```python
from build123d import *

# Parameters (mm, degrees)
SKETCH_1_R          = 10
EXTRUDE_1_DEPTH     = 377.5
SKETCH_2_W          = 20.903935991
SKETCH_2_H          = 21
CUT_EXTRUDE_1_DEPTH = 25
CUT_EXTRUDE_START   = -30
SKETCH_5_R          = 10
SKETCH_5_R_2        = 9.5
CUT_EXTRUDE_2_DEPTH = 1.1


with BuildPart() as part:
    # 草图1 → 凸台-拉伸1 (new, symmetric)
    with BuildSketch(Plane.XY):
        Circle(SKETCH_1_R)
    extrude(amount=EXTRUDE_1_DEPTH, both=True)

    # 草图2 → 切除-拉伸1 (cut, symmetric)
    with BuildSketch(Plane(origin=(0, 0, 0), x_dir=(1, 0, 0), z_dir=(0, 1, 0))):
        with Locations((-17.951967996, 367)):
            Rectangle(SKETCH_2_W, SKETCH_2_H)
        with Locations((17.951967996, 367)):
            Rectangle(SKETCH_2_W, SKETCH_2_H)
        with Locations((17.951967996, -367)):
            Rectangle(SKETCH_2_W, SKETCH_2_H)
        with Locations((-17.951967996, -367)):
            Rectangle(SKETCH_2_W, SKETCH_2_H)
    extrude(amount=CUT_EXTRUDE_1_DEPTH, both=True, mode=Mode.SUBTRACT)

    # 草图5 → 切除-拉伸2 (cut)
    with BuildSketch(Plane(origin=(0, 0, -377.5), x_dir=(-1, 0, 0), z_dir=(0, 0, -1)).offset(CUT_EXTRUDE_START)):
        Circle(SKETCH_5_R)
        Circle(SKETCH_5_R_2, mode=Mode.SUBTRACT)
    cut_extrude_2 = extrude(amount=CUT_EXTRUDE_2_DEPTH, mode=Mode.SUBTRACT)

    # 镜向1: 切除-拉伸2 across plane
    add(cut_extrude_2.mirror(Plane.XY), mode=Mode.SUBTRACT)


solid = part.part
```
The listing builds one solid part. Answer for the finished solid, in the listing's coordinates (mm). A direction names the side the tool comes from. Round coordinates to 2 decimals unless told otherwise and drop trailing zeros. Loops run counter-clockwise (first coordinate to the right, second up) from the corner with the lowest first, then second, coordinate; pieces in that order, holes last.
1) Consider line 1 (Z direction, x = -4.25, y = -8.75); line 2 (Y direction, x = -0.5, z = 44); line 3 (X direction, y = -7.5, z = -194.5). Determine where each line is inside the solid, lowest interval first.
Outcome:
line 1: z = -377.5 to -348.6, -347.5 to 347.5, 348.6 to 377.5
line 2: y = -9.99 to 9.99
line 3: x = -6.61 to 6.61
2) For faces 4 (the face through (-4.38, -8.43, -348.04)), 5 (the face through (7.5, 0, 367)), 6 (the face through (-7.5, 0, 367)), 7 (the face through (7.5, 0, -367)), determine the directions among +Z, -Z, +X, -X, +Y, -Y from which every point of the face is accessible in a straight line to the end or side of a thin tool.
Outcome:
face 4: none
face 5: +Z, +X, +Y, -Y
face 6: +Z, -X, +Y, -Y
face 7: -Z, +X, +Y, -Y
3) Given P1, Ø10.5, axis at y = -2, z = 371, coming from the -X side; P2, Ø4, axis at x = 4.5, z = 75.5, coming from the -Y side; P3, Ø6.5, axis at y = -2.5, z = 369.5, coming from the +X side; P4, Ø12, axis at x = -4.5, z = 13.5, coming from the -Y side, each flat-ended and moving along its own axis, determine where each tip first touches the part or whether it passes through.
Outcome:
P1: stops at x = -7.5
P2: stops at y = -9.68
P3: stops at x = 7.5
P4: stops at y = -10
4) A cutting plane is placed at A-A on x = 3.5. Determine the outline of the cut face in (y, z).
Outcome:
outline: (-9.37, -377.5) - (9.37, -377.5) - (9.37, -348.6) - (8.83, -348.6) - (8.83, -347.5) - (9.37, -347.5) - (9.37, 347.5) - (8.83, 347.5) - (8.83, 348.6) - (9.37, 348.6) - (9.37, 377.5) - (-9.37, 377.5) - (-9.37, 348.6) - (-8.83, 348.6) - (-8.83, 347.5) - (-9.37, 347.5) - (-9.37, -347.5) - (-8.83, -347.5) - (-8.83, -348.6) - (-9.37, -348.6) - close
5) For a pull along Z with two mould halves and no side action, classify faces 1 (the face through (0, 0, 377.5)), 2 (the face through (0, 0, -377.5)), 3 (the face through (-9, -4, -347.5)) as released by +Z, released by -Z, zero draft, split by the parting line, or undercut.
Outcome:
face 1: released by +Z
face 2: released by -Z
face 3: undercut
6) A cutting plane is placed at B-B on z = 326.5. Determine the outline of the cut face in (x, y), plus the area to 3 significant figures.
Outcome:
outline: circle Ø20 at (0, 0)
area: 314 mm2
